from build123d import *

# Parameters (mm, degrees)
ANGLED_BRACKET_BODY_DEPTH  = 25
SLOT_20X5_SKETCH_W         = 83.357534166
SLOT_20X5_SKETCH_H         = 20
SLOT_CUT_20X5_DEPTH        = 6
POCKET_CUT_28X14_DEPTH     = 6
RECESS_40X10_SKETCH_W      = 40
RECESS_40X10_SKETCH_H      = 10
RECESS_CUT_40X10_DEPTH     = 10
CLEVIS_BLOCK_SKETCH_W      = 36
CLEVIS_BLOCK_SKETCH_H      = 28
CLEVIS_BLOCK_DEPTH         = 50
PIVOT_BOSSES_DEPTH         = 10
PIVOT_BOSSES_DEPTH_BACK    = 60
PIVOT_BOSS_SKETCH_R        = 18
CLEVIS_SLOT_SKETCH_W       = 20
CLEVIS_SLOT_SKETCH_H       = 46
CLEVIS_SLOT_20_WIDE_DEPTH  = 80
PIVOT_BORE_SKETCH_R        = 9
PIVOT_BORE_18_DEPTH        = 80
MOUNTING_HOLES_SKETCH_R    = 6
MOUNTING_HOLES_2X_12_DEPTH = 39


with BuildPart() as part:
    # Bracket Profile Sketch → Angled Bracket Body (new, symmetric)
    with BuildSketch(Plane.XY):
        with BuildLine():
            Line((125, 0), (0, 0))
            Line((0, 0), (-42.5, 73.612159322))
            Line((-42.5, 73.612159322), (26.782032303, 113.612159322))
            Line((26.782032303, 113.612159322), (32.020529704, 105.094052432))
            Line((32.020529704, 105.094052432), (-20.181419095, 74.955243241))
            ThreePointArc((-20.181419095, 74.955243241), (-22.511048226, 71.919211448), (-22.011546114, 68.125116222))
            Line((-22.011546114, 68.125116222), (7.216878365, 17.5))
            ThreePointArc((7.216878365, 17.5), (9.047005384, 15.669872981), (11.547005384, 15))
            Line((11.547005384, 15), (125, 15))
            Line((125, 15), (125, 0))
        make_face()
    extrude(amount=ANGLED_BRACKET_BODY_DEPTH, both=True)

    # Slot 20x5 Sketch → Slot Cut 20x5 (cut)
    with BuildSketch(Plane(origin=(-42.5, 73.612159322, 0), x_dir=(0.8660254037844364, 0.5000000000000041, 0), z_dir=(-0.5000000000000041, 0.8660254037844364, 0))):
        with Locations((46.678767083, 0)):
            Rectangle(SLOT_20X5_SKETCH_W, SLOT_20X5_SKETCH_H)
    extrude(amount=-SLOT_CUT_20X5_DEPTH, mode=Mode.SUBTRACT)

    # Pocket 28x14 Sketch → Pocket Cut 28x14 (cut)
    with BuildSketch(Plane(origin=(-42.5, 73.612159322, 0), x_dir=(0.8660254037844364, 0.5000000000000041, 0), z_dir=(-0.5000000000000041, 0.8660254037844364, 0))):
        Polygon((0, 14), (0, -14), (5, -10), (5, 10), align=None)
    extrude(amount=-POCKET_CUT_28X14_DEPTH, mode=Mode.SUBTRACT)

    # Recess 40x10 Sketch → Recess Cut 40x10 (cut)
    with BuildSketch(Plane(origin=(-39.5, 68.416006899, 0), x_dir=(0.8660254037844364, 0.5000000000000041, 0), z_dir=(-0.500000000000004, 0.8660254037844363, 0))):
        with Locations((50, 0)):
            Rectangle(RECESS_40X10_SKETCH_W, RECESS_40X10_SKETCH_H)
    extrude(amount=-RECESS_CUT_40X10_DEPTH, mode=Mode.SUBTRACT)

    # Clevis Block Sketch → Clevis Block (add)
    with BuildSketch(Plane(origin=(100, 0, 0), x_dir=(0, 0, -1), z_dir=(1, 0, 0))):
        with Locations((0, 29)):
            Rectangle(CLEVIS_BLOCK_SKETCH_W, CLEVIS_BLOCK_SKETCH_H)
    extrude(amount=-CLEVIS_BLOCK_DEPTH)

    # Pivot Boss Sketch → Pivot Bosses (add, two sides: drawn at the far end of the back side and taken through both)
    with BuildSketch(Plane(origin=(100, 0, 0), x_dir=(0, 0, -1), z_dir=(1, 0, 0)).offset(-PIVOT_BOSSES_DEPTH_BACK)):
        with Locations((0, 43)):
            Circle(PIVOT_BOSS_SKETCH_R)
    extrude(amount=PIVOT_BOSSES_DEPTH + PIVOT_BOSSES_DEPTH_BACK)

    # Clevis Slot Sketch → Clevis Slot 20 Wide (cut)
    with BuildSketch(Plane.XY.offset(18)):
        with Locations((75, 43)):
            Rectangle(CLEVIS_SLOT_SKETCH_W, CLEVIS_SLOT_SKETCH_H)
    extrude(amount=-CLEVIS_SLOT_20_WIDE_DEPTH, mode=Mode.SUBTRACT)

    # Pivot Bore Sketch → Pivot Bore Ø18 (cut)
    with BuildSketch(Plane(origin=(110, 0, 0), x_dir=(0, 0, -1), z_dir=(1, 0, 0))):
        with Locations((0, 43)):
            Circle(PIVOT_BORE_SKETCH_R)
    extrude(amount=-PIVOT_BORE_18_DEPTH, mode=Mode.SUBTRACT)

    # Mounting Holes Sketch → Mounting Holes 2xØ12 (cut)
    with BuildSketch(Plane(origin=(0, 0, 0), x_dir=(0, 0, 1), z_dir=(-0.8660254037844363, -0.5000000000000042, 0))):
        with Locations(Location((0, 50, 0), (0, 0, 270))):
            Circle(MOUNTING_HOLES_SKETCH_R)
        with Locations(Location((0, 25, 0), (0, 0, 270))):
            Circle(MOUNTING_HOLES_SKETCH_R)
    extrude(amount=-MOUNTING_HOLES_2X_12_DEPTH, mode=Mode.SUBTRACT)


solid = part.part
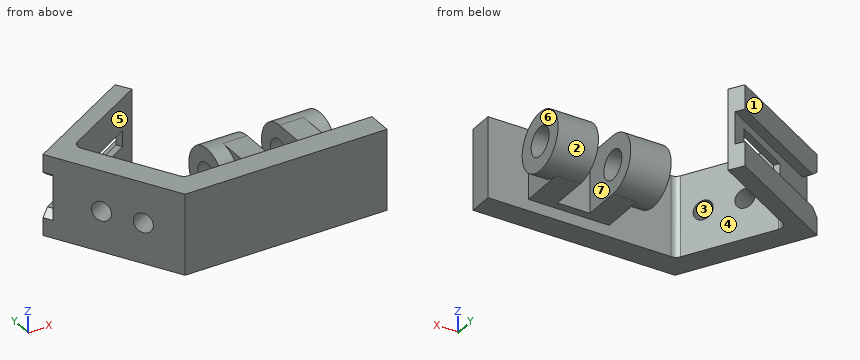
Check sheet for the modelled part. Datum: model origin and axes. Units: mm. Face numbers are marked on the shaded views. A direction names the side the tool comes from. Give positions to 0.01 mm unless a question says otherwise; leave off trailing zeros. Write each loop counter-clockwise with the first axis right and the second up, starting at its lowest first coordinate (ties: lowest second). Pieces come first, ordered by that corner, then holes. Notation, with made-up numbers: (-8, 71.5) -> (18, 71.5) arc R28 cw to (18, 99.5) -> close; hole circle Ø9 at (70, -20.75). An arc over 180 degrees is marked (long way). One line per item, written item: value. Start each with the question number.
Item 1: Section check C-C on z = 0. State how many separate pieces and enclosed holes the cut face has, then the cut area to 3 significant figures.
Item 2: Section check A-A on x = 58.5. Record the cut outline in (y, z).
Item 3: Material ranges on probe 1 along Y at (x, z) = (100.75, 0); probe 2 along X at (y, z) = (36, -15.5); probe 3 along Y at (x, z) = (99.75, 0), recorded low to high. Write a range as from..to.
Item 4: Draft check along Z on the marked faces 1, 2 and 3. Enter one of: +Z half, -Z half, draft (parallel to the pull), parting line (faces both ways), or undercut.
Item 5: Gauge pin test, flat ends, axial feed: pin 1 (22.5 mm diameter, centred on x = 70, y = 35, fed in from +Z); pin 2 (8.5 mm diameter, centred on y = 30, z = 2, fed in from +X); pin 3 (25 mm diameter, centred on x = 84.5, z = 11.5, fed in from +Y). Record the tip position at first contact, or that the pin passes through.
Item 6: Section check B-B on z = 20. Record the cut outline in (x, y), then the cut area to 3 significant figures.
Item 7: Tool access check on the marked faces 4, 5, 6 and 7. Record the directions out of +Z, -Z, +X, -X, +Y, -Y that give a thin tool (end or side, any length) a straight path to the whole face; none if there is none.
Results list:
1. separate pieces: 6
1. enclosed holes: 0
1. area: 3,980 mm²
2. outline: (0, -25) -> (15, -25) -> (15, -18) -> (43, -18) arc R18 ccw to (43, 18) -> (15, 18) -> (15, 25) -> (0, 25) -> close; hole circle Ø18 at (43, 0)
3. probe 1: 0..15, 25..34, 52..61
3. probe 2: -20.78..-3.46, 40..65, 85..110
3. probe 3: 0..34, 52..61
4. face 1: draft
4. face 2: parting line
4. face 3: undercut
5. pin 1: z = 18
5. pin 2: x = 110
5. pin 3: y = 61
6. outline: (-42.5, 73.61) -> (0, 0) -> (125, 0) -> (125, 15) -> (11.55, 15) arc R5 cw to (7.22, 17.5) -> (-22.01, 68.13) arc R5 cw to (-20.18, 74.96) -> (32.02, 105.09) -> (26.78, 113.61) -> close
6. area: 3,680 mm²
7. face 4: +Z, -Z
7. face 5: +Z, -Z, +X
7. face 6: +Z, -Z, +X, +Y
7. face 7: +Z, -Z, +Y
